```python
from build123d import *

# Parameters (mm, degrees)
BOSS_EXTRUDE1_DEPTH = 22
SKETCH2_W           = 2.8
SKETCH2_H           = 0.3
CUT_EXTRUDE1_DEPTH  = 5
SKETCH3_R           = 1.25
SKETCH3_R_2         = 1.05
CUT_EXTRUDE2_DEPTH  = 0.1
CUT_EXTRUDE3_DEPTH  = 0.1
SKETCH5_W           = 1.35
SKETCH5_H           = 5


with BuildPart() as part:
    # Sketch1 → Boss-Extrude1 (new body)
    with BuildSketch(Plane.XY):
        with BuildLine():
            Line((1.4, 1.428285686), (1.4, 2.5))
            Line((1.4, 2.5), (-1.4, 2.5))
            Line((-1.4, 2.5), (-1.4, 1.428285686))
            ThreePointArc((-1.4, 1.428285686), (0, -2), (1.4, 1.428285686))
        make_face()
    extrude(amount=-BOSS_EXTRUDE1_DEPTH)

    # Sketch2 → Cut-Extrude1 (cut)
    with BuildSketch(Plane.XY):
        with Locations((0, 2.35)):
            Rectangle(SKETCH2_W, SKETCH2_H)
    extrude(amount=-CUT_EXTRUDE1_DEPTH, mode=Mode.SUBTRACT)

    # Sketch3 → Cut-Extrude2 (cut)
    with BuildSketch(Plane(origin=(0, 2.2, 0), x_dir=(1, 0, 0), z_dir=(0, 1, 0))):
        with Locations(Location((0, 2, 0), (0, 0, 270))):
            Circle(SKETCH3_R)
        with Locations(Location((0, 2, 0), (0, 0, 270))):
            Circle(SKETCH3_R_2, mode=Mode.SUBTRACT)
    extrude(amount=-CUT_EXTRUDE2_DEPTH, mode=Mode.SUBTRACT)

    # Sketch4 → Cut-Extrude3 (cut)
    with BuildSketch(Plane(origin=(0, 2.2, 0), x_dir=(1, 0, 0), z_dir=(0, 1, 0))):
        with BuildLine():
            Line((-0.54433356, 1.10211305), (0.89788695, 2.54433356))
            ThreePointArc((0.89788695, 2.54433356), (0.74246212, 2.74246212), (0.54433356, 2.89788695))
            Line((0.54433356, 2.89788695), (-0.89788695, 1.45566644))
            ThreePointArc((-0.89788695, 1.45566644), (-0.74246212, 1.25753788), (-0.54433356, 1.10211305))
        make_face()
    extrude(amount=-CUT_EXTRUDE3_DEPTH, mode=Mode.SUBTRACT)

    # Sketch5 → Revolve1 (revolve)
    with BuildSketch(Plane(origin=(0, 0, 0), x_dir=(1, 0, 0), z_dir=(0, 1, 0)), mode=Mode.PRIVATE) as revolve1_sk:
        with Locations((-0.675, 24.5)):
            Rectangle(SKETCH5_W, SKETCH5_H)
    revolve(revolve1_sk.sketch.rotate(Axis((0, 0, -27), (0, 0, 1)), 180), axis=Axis((0, 0, -27), (0, 0, 1)))


solid = part.part
```
Input: part model. Units: mm. Frame: model coordinates. A direction names the side the tool comes from. Coordinates: 2 decimals unless noted, no trailing zeros. Loops run counter-clockwise (first coordinate to the right, second up) from the corner with the lowest first, then second, coordinate; pieces in that order, holes last. Notation, with made-up numbers: (6.5, 80) - (63.5, 80) arc R22 cw to (63.5, 103) - close; hole circle Ø8 at (-26, 84). An arc over 180 degrees is marked (long way). Answer in a Markdown table with one row per item.
(1) Set-up query: faces 1 (the face through (-1.4, 2, -11)), 2 (the face through (-1.07, -0.82, -24.54)), 3 (the face through (0, 2.2, -4)). Return all of +Z, -Z, +X, -X, +Y, -Y with unobstructed straight access to the full face (end or side cutting, diameter ignored); none if empty.
Model answer:
| item | result |
|---|---|
| face 1 | +Z, -Z, -X, +Y |
| face 2 | -Z |
| face 3 | +Z, +X, -X, +Y |
(2) Cut plane A-A on y = 0. Output: boundary loops of the cut face in (x, z).
Model answer:
| item | result |
|---|---|
| outline | (-2, -22) - (-1.35, -22) - (-1.35, -27) - (1.35, -27) - (1.35, -22) - (2, -22) - (2, 0) - (-2, 0) - close |
(3) Cut plane B-B on z = -15.5. Output: boundary loops of the cut face in (x, y), plus the area to 3 significant figures.
Model answer:
| item | result |
|---|---|
| outline | (-1.4, 1.43) arc R2 ccw (long way) to (1.4, 1.43) - (1.4, 2.5) - (-1.4, 2.5) - close |
| area | 14.5 mm² |
(4) Material intervals for L1, parallel to Z at x = -1.5, y = -1.25; L2, parallel to X at y = 2.15, z = -2; L3, parallel to Z at x = 0, y = 2.25, sorted ascending. Write a range as from..to.
Model answer:
| item | result |
|---|---|
| L1 | z = -22..0 |
| L2 | x = -1.4..-1.25, -1.05..-0.35, 0.35..1.05, 1.25..1.4 |
| L3 | z = -22..-5 |
(5) Cut plane C-C on x = 0. Output: boundary loops of the cut face in (y, z), plus the area to 3 significant figures.
Model answer:
| item | result |
|---|---|
| outline | (-2, -22) - (-1.35, -22) - (-1.35, -27) - (1.35, -27) - (1.35, -22) - (2.5, -22) - (2.5, -5) - (2.2, -5) - (2.2, -3.25) - (2.1, -3.25) - (2.1, -3.05) - (2.2, -3.05) - (2.2, -2.35) - (2.1, -2.35) - (2.1, -1.65) - (2.2, -1.65) - (2.2, -0.95) - (2.1, -0.95) - (2.1, -0.75) - (2.2, -0.75) - (2.2, 0) - (-2, 0) - close |
| area | 111 mm² |
(6) Pin query (flat end, axial travel): P1, Ø0.5, axis at x = -0.5, z = -2.5, coming from the +Y side; P2, Ø0.5, axis at y = 2, z = -11.5, coming from the +X side. Return the tip coordinate at first contact, or that it passes through.
Model answer:
| item | result |
|---|---|
| P1 | stops at y = 2.2 |
| P2 | stops at x = 1.4 |
(7) Mould query, pull axis Z, two halves, no side actions, for faces 4 (the face through (-0.4, 2.2, -2.4)), 5 (the face through (0, 0, -27)), 6 (the face through (0, 2.1, -2)). Classes: pulls with the +Z half, pulls with the -Z half, needs draft (parallel to the pull), parting line crosses it, or undercut.
Model answer:
| item | result |
|---|---|
| face 4 | needs draft |
| face 5 | pulls with the -Z half |
| face 6 | undercut |
(8) Cut plane D-D on z = -23.25. Output: boundary loops of the cut face in (x, y), plus the area to 3 significant figures.
Model answer:
| item | result |
|---|---|
| outline | circle Ø2.7 at (0, 0) |
| area | 5.73 mm² |
